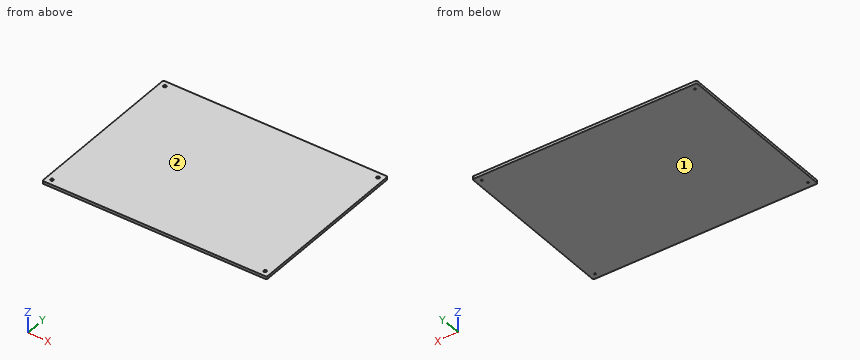
```python
from build123d import *

# Parameters (mm, degrees)
SKETCH_1_W                   = 800
SKETCH_1_H                   = 600
EXTRUDE_1_DEPTH              = 10
HOLE_WIZARD_M6_1_D           = 6.6
HOLE_WIZARD_M6_1_CBORE_D     = 11
HOLE_WIZARD_M6_1_CBORE_DEPTH = 6.4
FILLET_1_R                   = 5


with BuildPart() as part:
    # 草图1 → 凸台-拉伸1 (new body)
    with BuildSketch(Plane.XY):
        Rectangle(SKETCH_1_W, SKETCH_1_H)
    extrude(amount=EXTRUDE_1_DEPTH)

    # M6 六角凹头螺钉的柱形沉头孔1 (through all)
    with Locations(Plane.XY.offset(10)):
        with Locations((-380, 280), (380, 280), (380, -280), (-380, -280)):
            CounterBoreHole(HOLE_WIZARD_M6_1_D / 2, HOLE_WIZARD_M6_1_CBORE_D / 2, HOLE_WIZARD_M6_1_CBORE_DEPTH)

    # 圆角1
    fillet_1_edges = [part.edges().sort_by_distance(p)[0] for p in [
        (400, -300, 5),
        (-400, -300, 5),
        (-400, 300, 5),
        (400, 300, 5),
    ]]
    fillet(fillet_1_edges, radius=FILLET_1_R)


solid = part.part
```
For this review, take the finished solid that the model builds, in its own axes (mm). Face numbers are marked on the shaded views. Coordinates: 2 decimals unless noted, no trailing zeros. Answer in a Markdown table with one row per item. Add a question column.
Q1. Draft analysis for pull direction Z (two halves, no side actions). For the marked faces 1 and 2, state which applies: +Z half, -Z half, draft (parallel to the pull), parting line (faces both ways), or undercut.
Q2. For probe 1 along X at (y, z) = (-280, 7); probe 2 along Y at (x, z) = (-380, 1.25); probe 3 along X at (y, z) = (280, 2.6), list the stretches that pass through material, from the lowest coordinate up.
Q3. For P1, Ø17.5, axis at x = 380, y = 280, coming from the +Z side; P2, Ø5.5, axis at x = -380.5, y = -279, coming from the +Z side; P3, Ø6.5, axis at x = 380, y = -280, coming from the -Z side, all flat-tipped, find the tip position at first contact; note any pin that passes through.
Answer list:
| question | item | result |
|---|---|---|
| 1 | face 1 | -Z half |
| 1 | face 2 | +Z half |
| 2 | probe 1 | x = -400 to -385.5, -374.5 to 374.5, 385.5 to 400 |
| 2 | probe 2 | y = -300 to -283.3, -276.7 to 276.7, 283.3 to 300 |
| 2 | probe 3 | x = -400 to -383.3, -376.7 to 376.7, 383.3 to 400 |
| 3 | P1 | stops at z = 10 |
| 3 | P2 | stops at z = 3.6 |
| 3 | P3 | passes through |
